Could you check a few things on this model? Use its own coordinates, in mm. A direction names the side the tool comes from. Round coordinates to 2 decimals unless told otherwise and drop trailing zeros. Loops run counter-clockwise (first coordinate to the right, second up) from the corner with the lowest first, then second, coordinate; pieces in that order, holes last. Notation, with made-up numbers: (23, 75) -> (34, 75) arc R24 ccw to (34, 112) -> close; hole circle Ø6 at (57, -27). An arc over 180 degrees is marked (long way). Write each question's results on one line, items separated by ' | '.
from build123d import *

# Parameters (mm, degrees)
SKETCH1_W               = 400
SKETCH1_H               = 200
BOSS_EXTRUDE1_DEPTH     = 15
SKETCH2_R               = 6.5
CUT_EXTRUDE1_DEPTH      = 9
LPATTERN1_COUNT         = 3
LPATTERN1_PITCH         = 75
MIRROR1_COPY_1_SKETCH_R = 6.5
MIRROR1_COPY_1_DEPTH    = 9
MIRROR1_COPY_2_SKETCH_R = 6.5
MIRROR1_COPY_2_DEPTH    = 9
SKETCH3_R               = 4.5
CUT_EXTRUDE2_DEPTH      = 85
LPATTERN2_COUNT         = 3
LPATTERN2_PITCH         = 75
MIRROR2_COPY_1_SKETCH_R = 4.5
MIRROR2_COPY_1_DEPTH    = 85
MIRROR2_COPY_2_SKETCH_R = 4.5
MIRROR2_COPY_2_DEPTH    = 85
SKETCH4_R               = 6.5
CUT_EXTRUDE3_DEPTH      = 85
LPATTERN3_COUNT         = 3
LPATTERN3_PITCH         = 130
SKETCH5_R               = 5.5
CUT_EXTRUDE4_DEPTH      = 51
LPATTERN4_COUNT         = 3
LPATTERN4_PITCH         = 110


with BuildPart() as part:
    # Sketch1 → Boss-Extrude1 (new body)
    with BuildSketch(Plane.XY):
        Rectangle(SKETCH1_W, SKETCH1_H)
    extrude(amount=BOSS_EXTRUDE1_DEPTH)

    # Sketch2 → Cut-Extrude1 (cut)
    with BuildSketch(Plane.XY.offset(15)):
        with Locations((-192.5, 75)):
            Circle(SKETCH2_R)
    cut_extrude1 = extrude(amount=-CUT_EXTRUDE1_DEPTH, mode=Mode.SUBTRACT)

    # LPattern1: Cut-Extrude1 ×3
    with Locations(*[(0, -i * LPATTERN1_PITCH, 0) for i in range(1, LPATTERN1_COUNT)]):
        add(cut_extrude1, mode=Mode.SUBTRACT)

    # Mirror1: Cut-Extrude1 across plane
    add(cut_extrude1.mirror(Plane(origin=(0, 0, 0), x_dir=(0, 0, 1), z_dir=(1, 0, 0))), mode=Mode.SUBTRACT)

    # Mirror1 copy 1 sketch → Mirror1 copy 1 (cut)
    with BuildSketch(Plane(origin=(0, -75, 15), x_dir=(-1, 0, 0), z_dir=(0, 0, 1))):
        with Locations((-192.5, -75)):
            Circle(MIRROR1_COPY_1_SKETCH_R)
    extrude(amount=-MIRROR1_COPY_1_DEPTH, mode=Mode.SUBTRACT)

    # Mirror1 copy 2 sketch → Mirror1 copy 2 (cut)
    with BuildSketch(Plane(origin=(0, -150, 15), x_dir=(-1, 0, 0), z_dir=(0, 0, 1))):
        with Locations((-192.5, -75)):
            Circle(MIRROR1_COPY_2_SKETCH_R)
    extrude(amount=-MIRROR1_COPY_2_DEPTH, mode=Mode.SUBTRACT)

    # Sketch3 → Cut-Extrude2 (cut)
    with BuildSketch(Plane.XY.offset(15)):
        with Locations((-192.5, 75)):
            Circle(SKETCH3_R)
    cut_extrude2 = extrude(amount=-CUT_EXTRUDE2_DEPTH, mode=Mode.SUBTRACT)

    # LPattern2: Cut-Extrude2 ×3
    with Locations(*[(0, -i * LPATTERN2_PITCH, 0) for i in range(1, LPATTERN2_COUNT)]):
        add(cut_extrude2, mode=Mode.SUBTRACT)

    # Mirror2: Cut-Extrude2 across plane
    add(cut_extrude2.mirror(Plane(origin=(0, 0, 0), x_dir=(0, 0, 1), z_dir=(1, 0, 0))), mode=Mode.SUBTRACT)

    # Mirror2 copy 1 sketch → Mirror2 copy 1 (cut)
    with BuildSketch(Plane(origin=(0, -75, 15), x_dir=(-1, 0, 0), z_dir=(0, 0, 1))):
        with Locations((-192.5, -75)):
            Circle(MIRROR2_COPY_1_SKETCH_R)
    extrude(amount=-MIRROR2_COPY_1_DEPTH, mode=Mode.SUBTRACT)

    # Mirror2 copy 2 sketch → Mirror2 copy 2 (cut)
    with BuildSketch(Plane(origin=(0, -150, 15), x_dir=(-1, 0, 0), z_dir=(0, 0, 1))):
        with Locations((-192.5, -75)):
            Circle(MIRROR2_COPY_2_SKETCH_R)
    extrude(amount=-MIRROR2_COPY_2_DEPTH, mode=Mode.SUBTRACT)

    # Sketch4 → Cut-Extrude3 (cut)
    with BuildSketch(Plane.XY.offset(15)):
        with Locations((-130, 0)):
            Circle(SKETCH4_R)
    cut_extrude3 = extrude(amount=-CUT_EXTRUDE3_DEPTH, mode=Mode.SUBTRACT)

    # LPattern3: Cut-Extrude3 ×3
    with Locations(*[(i * LPATTERN3_PITCH, 0, 0) for i in range(1, LPATTERN3_COUNT)]):
        add(cut_extrude3, mode=Mode.SUBTRACT)

    # Sketch5 → Cut-Extrude4 (cut)
    with BuildSketch(Plane.XY.offset(15)):
        with Locations((-75, 80)):
            Circle(SKETCH5_R)
    cut_extrude4 = extrude(amount=-CUT_EXTRUDE4_DEPTH, mode=Mode.SUBTRACT)

    # LPattern4: Cut-Extrude4 ×3
    with Locations(*[(i * LPATTERN4_PITCH, 0, 0) for i in range(1, LPATTERN4_COUNT)]):
        add(cut_extrude4, mode=Mode.SUBTRACT)


solid = part.part
1) I want a section at D-D, the plane x = 145. Write out the boundary of the cut face in (y, z).
Model answer:
outline: (-100, 0) -> (74.5, 0) -> (74.5, 15) -> (-100, 15) -> close; (85.5, 0) -> (100, 0) -> (100, 15) -> (85.5, 15) -> close
2) I want a section at B-B, the plane y = 0. Give the number of separate pieces and of enclosed holes in the cut face, plus the area to 3 significant figures.
Model answer:
separate pieces: 6 | enclosed holes: 0 | area: 5,070 mm2
3) For faces 1 (the cylindrical face through (197.658, 71.045, 10.563)), 2 (the cylindrical face through (188.34, 1.72, 3.04)), which set-ups out of +Z, -Z, +X, -X, +Y, -Y let a thin tool reach every point of the face, with its end or its side?
Model answer:
face 1: +Z | face 2: +Z, -Z
4) I want a section at A-A, the plane x = -130. Write out the boundary of the cut face in (y, z), plus the area to 4 significant figures.
Model answer:
outline: (-100, 0) -> (-6.5, 0) -> (-6.5, 15) -> (-100, 15) -> close; (6.5, 0) -> (100, 0) -> (100, 15) -> (6.5, 15) -> close | area: 2,805 mm2
5) If we mould it in two halves opening along X, with no side actions, what happens to faces 3 (the flat face through (-200, -1, 7)), 4 (the flat face through (-3, 24, 0)), 5 (the cylindrical face through (199, 0, 11))? For each: released by +X, released by -X, zero draft, split by the parting line, or undercut.
Model answer:
face 3: released by -X | face 4: zero draft | face 5: undercut
6) I'm going to push flat-ended pins straight in: pin 1 (11.5 mm diameter, centred on x = -130, y = 0, fed in from +Z); pin 2 (6.5 mm diameter, centred on x = -189.5, y = 76, fed in from +Z). Where does each tip first touch, or does it pass through?
Model answer:
pin 1: passes through | pin 2: stops at z = 6
7) I need wall thicknesses on line 1 (Y direction, x = 192.5, z = 12.5); line 2 (X direction, y = 2.5, z = 5.5); line 3 (X direction, y = -80.5, z = 13.75). Which ranges of each line are inside material? Lowest first, please.
Model answer:
line 1: y = -100 to -81.5, -68.5 to -6.5, 6.5 to 68.5, 81.5 to 100 | line 2: x = -200 to -196.24, -188.76 to -136, -124 to -6, 6 to 124, 136 to 188.76, 196.24 to 200 | line 3: x = -200 to -195.96, -189.04 to 189.04, 195.96 to 200
